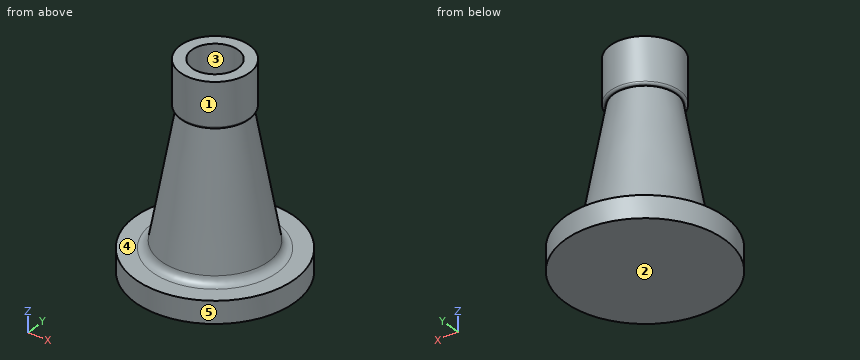
from build123d import *

# Parameters (mm, degrees)
FLANGE_SKETCH_145_R                = 72.5
FLANGE_145X20_DEPTH                = 20
TAPER_SKETCH_100_R                 = 50
TAPERED_BODY_100_10DEG_DRAFT_DEPTH = 125
TAPERED_BODY_100_10DEG_DRAFT_TAPER = 10
SPIGOT_63X38_DEPTH                 = 38
SPIGOT_63X38_DEPTH_BACK            = 3
SPIGOT_SKETCH_63_R                 = 31.5
BORE_SKETCH_42_R                   = 21
BORE_42X158_DEPTH                  = 158
FLANGE_ROOT_FILLET_R8_R            = 8
SPIGOT_EDGE_FILLET_R2_R            = 2


with BuildPart() as part:
    # Flange Sketch Ø145 → Flange Ø145x20 (new body)
    with BuildSketch(Plane.XY):
        Circle(FLANGE_SKETCH_145_R)
    extrude(amount=FLANGE_145X20_DEPTH)

    # Taper Sketch Ø100 → Tapered Body Ø100 10deg Draft (add)
    with BuildSketch(Plane.XY.offset(20)):
        Circle(TAPER_SKETCH_100_R)
    extrude(amount=TAPERED_BODY_100_10DEG_DRAFT_DEPTH, taper=TAPERED_BODY_100_10DEG_DRAFT_TAPER)

    # Spigot Sketch Ø63 → Spigot Ø63x38 (add, two sides: drawn at the far end of the back side and taken through both)
    with BuildSketch(Plane.XY.offset(145).offset(-SPIGOT_63X38_DEPTH_BACK)):
        Circle(SPIGOT_SKETCH_63_R)
    extrude(amount=SPIGOT_63X38_DEPTH + SPIGOT_63X38_DEPTH_BACK)

    # Bore Sketch Ø42 → Bore Ø42x158 (cut)
    with BuildSketch(Plane.XY.offset(183)):
        Circle(BORE_SKETCH_42_R)
    extrude(amount=-BORE_42X158_DEPTH, mode=Mode.SUBTRACT)

    # Flange Root Fillet R8
    flange_root_fillet_r8_edges = [part.edges().sort_by_distance(p)[0] for p in [
        (-50, 0, 20),
    ]]
    fillet(flange_root_fillet_r8_edges, radius=FLANGE_ROOT_FILLET_R8_R)

    # Spigot Edge Fillet R2
    spigot_edge_fillet_r2_edges = [part.edges().sort_by_distance(p)[0] for p in [
        (-31.5, 0, 142),
    ]]
    fillet(spigot_edge_fillet_r2_edges, radius=SPIGOT_EDGE_FILLET_R2_R)


solid = part.part
The listing builds one solid part. Answer for the finished solid, in the listing's coordinates (mm). Face numbers are marked on the shaded views. A direction names the side the tool comes from. Give positions to 0.01 mm unless a question says otherwise; leave off trailing zeros. Write each loop counter-clockwise with the first axis right and the second up, starting at its lowest first coordinate (ties: lowest second). Pieces come first, ordered by that corner, then holes.
1) A tool of negligible diameter and unlimited length cuts with its end or side. For the marked faces 4 and 5, from which of +Z, -Z, +X, -X, +Y, -Y can it reach the whole face along a straight path? Write none if from no direction.
2) Section A-A (x = 0) is taken. Write down the section's boundary in (y, z).
3) Section B-B (z = 54.5) is taken. Write down the section's boundary in (x, y), and give its area (3 significant figures).
4) Given P1, Ø3, axis at y = 25.5, z = 39, coming from the +X side; P2, Ø12, axis at x = 8, z = 111.5, coming from the -Y side; P3, Ø8, axis at x = -33, z = 31.5, coming from the +Y side; P4, Ø8, axis at x = -42, y = 29, coming from the -Z side, each flat-ended and moving along its own axis, determine where each tip first touches the part or whether it passes through.
5) Find the intervals of material crossed by L1, parallel to X at y = -11, z = 132; L2, parallel to Y at x = 0, z = 67.5; L3, parallel to Y at x = 0, z = 58, in increasing order.
6) For a pull along Y with two mould halves and no side action, classify the marked faces 1, 2 and 3 as pulls with the +Y half, pulls with the -Y half, needs draft (parallel to the pull), parting line crosses it, or undercut.
7) Section D-D (z = 107) is taken. Write down the section's boundary in (x, y).
Response:
1. face 4: +Z
1. face 5: +Z, -Z
2. outline: (-72.5, 0) - (72.5, 0) - (72.5, 20) - (56.71, 20) arc R8 cw to (48.83, 26.61) - (28.49, 142) - (29.5, 142) arc R2 ccw to (31.5, 144) - (31.5, 183) - (21, 183) - (21, 25) - (-21, 25) - (-21, 183) - (-31.5, 183) - (-31.5, 144) arc R2 ccw to (-29.5, 142) - (-28.49, 142) - (-48.83, 26.61) arc R8 cw to (-56.71, 20) - (-72.5, 20) - close
3. outline: circle Ø87.83 at (0, 0); hole circle Ø42 at (0, 0)
3. area: 4,670 mm2
4. P1: stops at x = 40.05
4. P2: stops at y = -34.43
4. P3: stops at y = 38.34
4. P4: stops at z = 0
5. L1: x = -28.18 to -17.89, 17.89 to 28.18
5. L2: y = -41.62 to -21, 21 to 41.62
5. L3: y = -43.3 to -21, 21 to 43.3
6. face 1: parting line crosses it
6. face 2: needs draft
6. face 3: undercut
7. outline: circle Ø69.32 at (0, 0); hole circle Ø42 at (0, 0)
